Could you check a few things on this model? Use its own coordinates, in mm. A direction names the side the tool comes from. Give positions to 0.01 mm unless a question says otherwise; leave off trailing zeros. Loops run counter-clockwise (first coordinate to the right, second up) from the corner with the lowest first, then second, coordinate; pieces in that order, holes last. Notation, with made-up numbers: M 86.5,2 L 91.5,2 A28 ccw 91.5,32 Z; hole C -17,59.5 d5. An arc over 180 degrees is marked long. Use a Markdown table: item, result. Add a question column.
1) If I drill on line 1 along Y through (x, z) = (35.5, 13.5); line 2 along Y through (x, z) = (80, 5); line 3 along Y through (x, z) = (19.5, 9), over which ranges is the centre line in solid material (lowest first)? Write a range as [from, to].
2) We'd pull the mould along X, two halves only. Please class faces 4 (the flat face through (5, 159, 10)), 5 (the flat face through (-1, 159, 10)), 6 (the flat face through (84, 173, 10)): +X half, -X half, draft (parallel to the pull), parting line (faces both ways), or undercut.
3) Will these pins go through, and if not, where does the flat tip stop? pin 1 Ø8 at (x, y) = (95, 24.5) entering from +Z; pin 2 Ø6 at (y, z) = (161.5, 8) entering from -X; pin 3 Ø10 at (y, z) = (159, 5.5) entering from +X.
4) Suppose I cut it at B-B on x = 102. List the corners of the cut face in (y, z) for me.
5) Suppose I cut it at A-A on z = 14.5. List the corners of the cut face in (x, y) for me.
6) Which directions (+Z, -Z, +X, -X, +Y, -Y) give clear straight access to the entire face, cutting with the end or side of a thin tool? Please do faces 1 (the flat face through (171, 159, 10)), 2 (the cylindrical face through (172.59, 2.62, 5.07)), 3 (the flat face through (84, 167, 10)).
7) Suppose I cut it at D-D on x = 80. List the corners of the cut face in (y, z) for me.
8) Suppose I cut it at C-C on y = 157. List the corners of the cut face in (x, z) for me, and give its area (3 significant figures).
```python
from build123d import *

# Parameters (mm, degrees)
SKETCH1_R           = 3
SKETCH1_R_2         = 4
BOSS_EXTRUDE1_DEPTH = 10
SKETCH2_W           = 192.506357526
SKETCH2_H           = 41.072090777
BOSS_EXTRUDE2_DEPTH = 10
FILLET1_R           = 10
SKETCH3_W           = 172
SKETCH3_H           = 27
SKETCH3_W_2         = 160
SKETCH3_H_2         = 15
BOSS_EXTRUDE3_DEPTH = 10


with BuildPart() as part:
    # Sketch1 → Boss-Extrude1 (new body)
    with BuildSketch(Plane.XY):
        Polygon((0, 0), (170, 0), (160, 146), (10, 146), align=None)
        with Locations((95, 24.5)):
            Circle(SKETCH1_R, mode=Mode.SUBTRACT)
        with Locations((80, 99.5)):
            Circle(SKETCH1_R_2, mode=Mode.SUBTRACT)
    extrude(amount=BOSS_EXTRUDE1_DEPTH)

    # Sketch2 → Boss-Extrude2 (add)
    with BuildSketch(Plane(origin=(0, 0, 0), x_dir=(-1, 0, 0), z_dir=(0, -1, 0))):
        with Locations((-84.638287431, -5.918559418)):
            Rectangle(SKETCH2_W, SKETCH2_H)
    extrude(amount=BOSS_EXTRUDE2_DEPTH)

    # Fillet1
    fillet1_edges = [part.edges().sort_by_distance(p)[0] for p in [
        (170, 0, 5),
        (0, 0, 5),
    ]]
    fillet(fillet1_edges, radius=FILLET1_R)

    # Sketch3 → Boss-Extrude3 (add, symmetric)
    with BuildSketch(Plane.XY.offset(10)):
        with Locations((85, 159.5)):
            Rectangle(SKETCH3_W, SKETCH3_H)
        with Locations((85, 159.5)):
            Rectangle(SKETCH3_W_2, SKETCH3_H_2, mode=Mode.SUBTRACT)
    extrude(amount=BOSS_EXTRUDE3_DEPTH, both=True)


solid = part.part
```
Answer block:
| question | item | result |
|---|---|---|
| 1 | line 1 | y = [-10, 0], [146, 152], [167, 173] |
| 1 | line 2 | y = [-10, 95.5], [103.5, 152], [167, 173] |
| 1 | line 3 | y = [-10, 152], [167, 173] |
| 2 | face 4 | undercut |
| 2 | face 5 | -X half |
| 2 | face 6 | draft |
| 3 | pin 1 | stops at z = 10 |
| 3 | pin 2 | stops at x = -1 |
| 3 | pin 3 | stops at x = 171 |
| 4 | outline | M -10,-14.62 L 0,-14.62 L 0,0 L 152,0 L 152,20 L 146,20 L 146,10 L 0,10 L 0,26.45 L -10,26.45 Z; M 167,0 L 173,0 L 173,20 L 167,20 Z |
| 5 | outline | M -11.61,-10 L 180.89,-10 L 180.89,0 L -11.61,0 Z; M -1,146 L 171,146 L 171,173 L -1,173 Z; hole M 5,152 L 165,152 L 165,167 L 5,167 Z |
| 6 | face 1 | +Z, -Z, +X, +Y |
| 6 | face 2 | +Z, -Z, +X |
| 6 | face 3 | +Z, -Z |
| 7 | outline | M -10,-14.62 L 0,-14.62 L 0,0 L 95.5,0 L 95.5,10 L 0,10 L 0,26.45 L -10,26.45 Z; M 103.5,0 L 152,0 L 152,20 L 146,20 L 146,10 L 103.5,10 Z; M 167,0 L 173,0 L 173,20 L 167,20 Z |
| 8 | outline | M -1,0 L 5,0 L 5,20 L -1,20 Z; M 165,0 L 171,0 L 171,20 L 165,20 Z |
| 8 | area | 240 mm^2 |
